```python
from build123d import *

# Parameters (mm, degrees)
SKETCH_1_R               = 40
EXTRUDE_1_DEPTH          = 50
SKETCH_2_W               = 6
SKETCH_2_H               = 20
EXTRUDE_2_DEPTH          = 16
CUT_EXTRUDE_1_DEPTH      = 89.345911054
PATTERN_CIRCULAR_1_COUNT = 3
SKETCH_4_R               = 8
CUT_EXTRUDE_2_DEPTH      = 87.925255248
PATTERN_CIRCULAR_2_COUNT = 3


with BuildPart() as part:
    # 草图1 → 凸台-拉伸1 (new body)
    with BuildSketch(Plane.XY):
        Circle(SKETCH_1_R)
    extrude(amount=EXTRUDE_1_DEPTH)

    # 草图2 → 凸台-拉伸2 (add)
    with BuildSketch(Plane.XY.offset(50)):
        with Locations((0, 18)):
            Rectangle(SKETCH_2_W, SKETCH_2_H)
    extrude_2 = extrude(amount=EXTRUDE_2_DEPTH)

    # 草图3 → 切除-拉伸1 (cut, through all)
    with BuildSketch(Plane.ZY.offset(3)):
        Polygon((54, 28), (54, 22), (60, 22), (60, 16), (66, 16), (66, 28), align=None)
    cut_extrude_1 = extrude(amount=-CUT_EXTRUDE_1_DEPTH, mode=Mode.SUBTRACT)

    # 阵列(圆周)1: 凸台-拉伸2, 切除-拉伸1 ×3 about axis
    pattern_circular_1_axis = Axis((0, 0, 0), (0, 0, 1))
    add([extrude_2.rotate(pattern_circular_1_axis, i * 360 / PATTERN_CIRCULAR_1_COUNT) for i in range(1, PATTERN_CIRCULAR_1_COUNT)])
    add([cut_extrude_1.rotate(pattern_circular_1_axis, i * 360 / PATTERN_CIRCULAR_1_COUNT) for i in range(1, PATTERN_CIRCULAR_1_COUNT)], mode=Mode.SUBTRACT)

    # 草图4 → 切除-拉伸2 (cut, through all)
    with BuildSketch(Plane(origin=(0, 0, 0), x_dir=(-1, 0, 0), z_dir=(0, 0, -1))):
        Circle(SKETCH_4_R)
    extrude(amount=-CUT_EXTRUDE_2_DEPTH, mode=Mode.SUBTRACT)

    # 草图5 → M6 螺纹孔1 (revolve, cut)
    with BuildSketch(Plane(origin=(0, 33, 0), x_dir=(0, 1, 0), z_dir=(1, 0, 0))):
        Polygon((0, 0), (0, 18.502151548), (2.5, 17), (2.5, 0), align=None)
    hole_wizard_m6_1 = revolve(axis=Axis((0, 33, -6.35), (0, 0, 1)), mode=Mode.SUBTRACT)

    # 阵列(圆周)2: M6 螺纹孔1 ×3 about axis
    pattern_circular_2_axis = Axis((0, 0, 0), (0, 0, 1))
    for i in range(1, PATTERN_CIRCULAR_2_COUNT):
        add(hole_wizard_m6_1.rotate(pattern_circular_2_axis, i * 360 / PATTERN_CIRCULAR_2_COUNT), mode=Mode.SUBTRACT)


solid = part.part
```
Design review of the part built by this model. Coordinates are the model's own, in mm. A direction names the side the tool comes from. Give positions to 0.01 mm unless a question says otherwise; leave off trailing zeros. Order: outer loops, then holes, each group sorted by start corner. A loop starts at its lowest first (then second) coordinate and runs counter-clockwise, first axis right, second up. Notation, with made-up numbers: M -1,83 L 22,83 A8 cw 22,90 Z; hole C 37,30 d10. An arc over 180 degrees is marked long. One line per question, with ' | ' between items. Start each with the question number.
Q1. For L1, parallel to Y at x = 0, z = 38; L2, parallel to X at y = -16.5, z = 4.5; L3, parallel to Z at x = 31.5, y = 15, list the stretches that pass through material, from the lowest coordinate up. Write a range as [from, to].
Q2. We need section A-A (y = 0). Write out the cut boundary in (x, z).
Q3. We need section C-C (x = -19.5). Write out the cut boundary in (y, z) (3 decimals).
Q4. The part is to be moulded in two halves that separate along X. For faces 4 (the face through (0, 16, 63)), 5 (the face through (-13.835, -8.036, 62.958)), 6 (the face through (-12.043, -10.417, 56.11)), say which applies: +X half, -X half, draft (parallel to the pull), parting line (faces both ways), or undercut.
Q5. Machinability: for faces 1 (the face through (-6.907, -4.036, 57.888)), 2 (the face through (30.1, -18.484, 8.381)), 3 (the face through (-3, 16, 56)), which of the approach directions +Z, -Z, +X, -X, +Y, -Y give a long, thin tool a straight path to every point of the face, cutting with its end or side? Answer none if there is none.
Q6. We need section D-D (z = 15). Write out the cut boundary in (x, y).
Q7. For pin 1 Ø9 at (x, y) = (-19.5, -12) entering from +Z; pin 2 Ø4 at (x, z) = (-23.5, 53) entering from +Y; pin 3 Ø4.5 at (x, z) = (0, 52) entering from +Y; pin 4 Ø9.5 at (x, y) = (0, 0) entering from -Z, all flat-tipped, find the tip position at first contact; note any pin that passes through.
Q8. We need section B-B (z = 22). Write out the cut boundary in (x, y), plus the area to 3 significant figures.
Returned:
1) L1: [-40, -8], [8, 40] | L2: [-36.44, -31.08], [-26.08, 26.08], [31.08, 36.44] | L3: [0, 50]
2) outline: M -40,0 L -8,0 L -8,50 L -40,50 Z; M 8,0 L 40,0 L 40,50 L 8,50 Z
3) outline: M -34.925,0 L 34.925,0 L 34.925,50 L -7.794,50 L -7.794,60 L -10.225,60 L -10.225,54 L -14.722,54 L -14.722,50 L -34.925,50 Z
4) face 4: draft | face 5: -X half | face 6: undercut
5) face 1: +Z, +Y | face 2: -Z | face 3: +Z, -X, +Y, -Y
6) outline: C 0,0 d80; hole C -28.58,-16.5 d5; hole C 0,0 d16; hole C 0,33 d5; hole C 28.58,-16.5 d5
7) pin 1: z = 60 | pin 2: y = -8.95 | pin 3: y = 40 | pin 4: through
8) outline: C 0,0 d80; hole C 0,0 d16 | area: 4,830 mm2
